Answer from the drawing. Dimensions are ordinates in mm from the lowest x, y and z of the part. A direction names the side the tool comes from. Coordinates: 2 decimals unless noted, no trailing zeros. Order: outer loops, then holes, each group sorted by start corner. A loop starts at its lowest first (then second) coordinate and runs counter-clockwise, first axis right, second up. Notation, with made-up numbers: (6.25, 34) -> (54.25, 34) arc R17 cw to (54.25, 66) -> close; hole circle Ø6 at (46, -9.5). An arc over 180 degrees is marked (long way). Use CSV: the item, a comma, the result in double quotes.
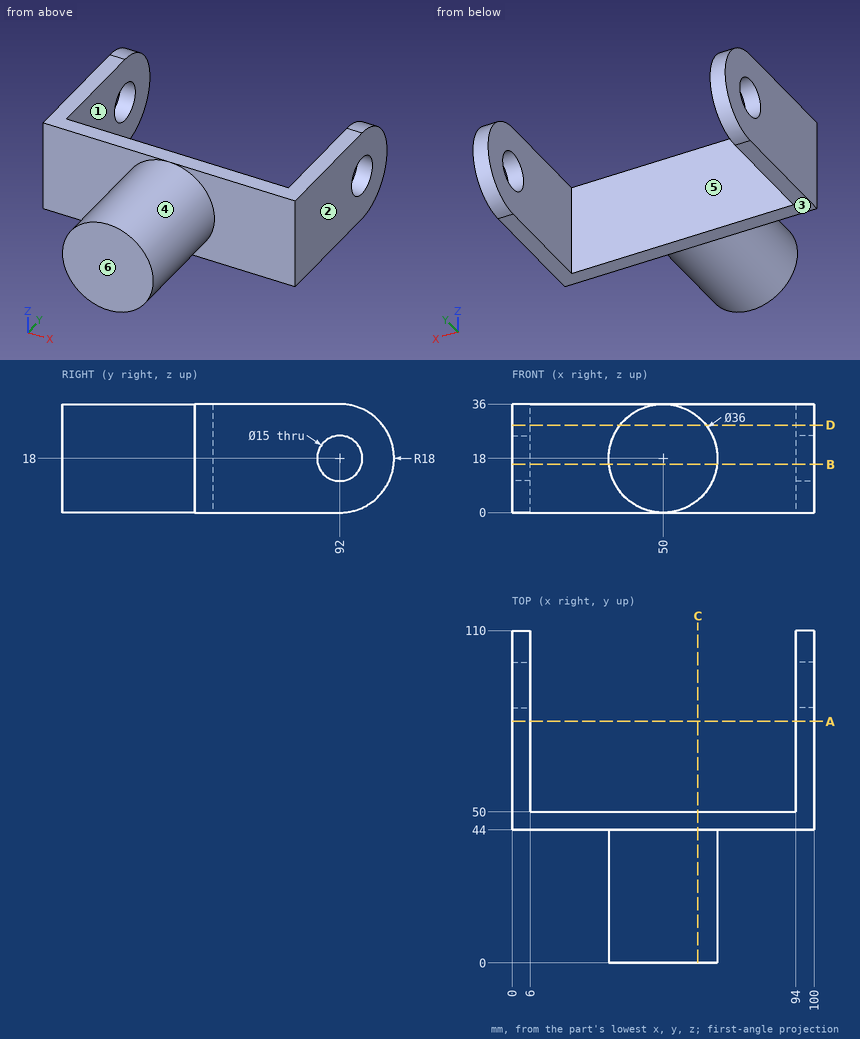
Item 1: The mould has two halves that part along X. Classify the marked faces 1, 2 and 3: +X half, -X half, draft (parallel to the pull), parting line (faces both ways), or undercut.
Return value:
face 1,"undercut"
face 2,"+X half"
face 3,"draft"
Item 2: A tool of negligible diameter and unlimited length cuts with its end or side. For the marked faces 4, 5 and 6, from which of +Z, -Z, +X, -X, +Y, -Y can it reach the whole face along a straight path? Write none if from no direction.
Return value:
face 4,"-Y"
face 5,"+Z, -Z, +Y"
face 6,"+Z, -Z, +X, -X, -Y"
Item 3: Straight lines are drawn through the part: line 1 along X through (y, z) = (71.5, 26.5); line 2 along Y through (x, z) = (1.95, 18); line 3 along Y through (x, z) = (38, 18.5). For each, find the intervals that lie inside material, in ascending order.
Return value:
line 1,"x = 0 to 6, 94 to 100"
line 2,"y = 44 to 84.5, 99.5 to 110"
line 3,"y = 0 to 50"
Item 4: Find section C-C, the plane x = 61.5. Give the vertices of the cut face in (y, z).
Return value:
outline,"(0, 4.15) -> (44, 4.15) -> (44, 0) -> (50, 0) -> (50, 36) -> (44, 36) -> (44, 31.85) -> (0, 31.85) -> close"
Item 5: Find section B-B, the plane z = 16. Give the vertices of the cut face in (x, y), then the cut area to 3 significant figures.
Return value:
outline,"(0, 44) -> (32.11, 44) -> (32.11, 0) -> (67.89, 0) -> (67.89, 44) -> (100, 44) -> (100, 84.77) -> (94, 84.77) -> (94, 50) -> (6, 50) -> (6, 84.77) -> (0, 84.77) -> close; (0, 99.23) -> (6, 99.23) -> (6, 109.89) -> (0, 109.89) -> close; (94, 99.23) -> (100, 99.23) -> (100, 109.89) -> (94, 109.89) -> close"
area,"2,720 mm^2"
Item 6: Find section D-D, the plane z = 29. Give the vertices of the cut face in (x, y), then the cut area to 3 significant figures.
Return value:
outline,"(0, 44) -> (35.75, 44) -> (35.75, 0) -> (64.25, 0) -> (64.25, 44) -> (100, 44) -> (100, 106.25) -> (94, 106.25) -> (94, 50) -> (6, 50) -> (6, 106.25) -> (0, 106.25) -> close"
area,"2,530 mm^2"
Item 7: Each of these flat-tipped pins is pushed along its axis until it touches: P1, Ø18, axis at x = 18.5, z = 24.5, coming from the -Y side; P2, Ø12, axis at x = 64, z = 26, coming from the +Y side; P3, Ø1.5, axis at y = 37.5, z = 16, coming from the +X side. Where does it stop, or does it pass through?
Return value:
P1,"stops at y = 44"
P2,"stops at y = 50"
P3,"stops at x = 67.96"
Item 8: Find section A-A, the plane y = 80. Give the vertices of the cut face in (x, z).
Return value:
outline,"(0, 0) -> (6, 0) -> (6, 36) -> (0, 36) -> close; (94, 0) -> (100, 0) -> (100, 36) -> (94, 36) -> close"
